from build123d import *

# Parameters (mm, degrees)
SKETCH_1_W      = 120
SKETCH_1_H      = 120
SKETCH_1_R      = 6.5
EXTRUDE_1_DEPTH = 10


with BuildPart() as part:
    # 草图1 → 凸台-拉伸1 (new body)
    with BuildSketch(Plane.XY):
        with Locations((60, 60)):
            Rectangle(SKETCH_1_W, SKETCH_1_H)
        with Locations((90, 35)):
            Circle(SKETCH_1_R, mode=Mode.SUBTRACT)
        with Locations((30, 85)):
            Circle(SKETCH_1_R, mode=Mode.SUBTRACT)
        with Locations((90, 85)):
            Circle(SKETCH_1_R, mode=Mode.SUBTRACT)
        with Locations((30, 35)):
            Circle(SKETCH_1_R, mode=Mode.SUBTRACT)
    extrude(amount=EXTRUDE_1_DEPTH)


solid = part.part
For this review, take the finished solid that the model builds, in its own axes (mm). Round coordinates to 2 decimals unless told otherwise and drop trailing zeros. Order: outer loops, then holes, each group sorted by start corner. A loop starts at its lowest first (then second) coordinate and runs counter-clockwise, first axis right, second up. Notation, with made-up numbers: (-27.75, 5.5) -> (7.25, 5.5) arc R27 cw to (7.25, 28.5) -> close; hole circle Ø5 at (43, -18). An arc over 180 degrees is marked (long way). Write item = value, one per line. Start each with the question number.
1) Take a section at C-C on z = 8. State the section outline as (x, y) points.
2) To check wall thickness, follow line 1 (Y direction, x = 30, z = 7.25); line 2 (Y direction, x = 84, z = 7); line 3 (X direction, y = 36.5, z = 8). State the ranges of each line that lie inside material, in increasing order. Write a range as from..to.
3) Take a section at A-A on x = 90. State the section outline as (y, z) points.
4) The part is to be moulded in two halves that separate along Y. For faces 1 (the face through (59, 0, 5)), 2 (the face through (28.591, 78.655, 4.93)), 3 (the face through (59, 120, 5)), say which applies: +Y half, -Y half, draft (parallel to the pull), parting line (faces both ways), or undercut.
5) Take a section at B-B on y = 85. State the section outline as (x, z) points, plus the area to 3 significant figures.
6) Insertion check: pin 1 (10.5 mm diameter, centred on x = 90, y = 85, fed in from -Z). The pin has a flat end and moves straight along its axis. Give the tip position at first contact, or say it passes through.
Verdict:
q1.outline = (0, 0) -> (120, 0) -> (120, 120) -> (0, 120) -> close; hole circle Ø13 at (30, 35); hole circle Ø13 at (30, 85); hole circle Ø13 at (90, 35); hole circle Ø13 at (90, 85)
q2.line_1 = 0..28.5, 41.5..78.5, 91.5..120
q2.line_2 = 0..32.5, 37.5..82.5, 87.5..120
q2.line_3 = 0..23.68, 36.32..83.68, 96.32..120
q3.outline = (0, 0) -> (28.5, 0) -> (28.5, 10) -> (0, 10) -> close; (41.5, 0) -> (78.5, 0) -> (78.5, 10) -> (41.5, 10) -> close; (91.5, 0) -> (120, 0) -> (120, 10) -> (91.5, 10) -> close
q4.face_1 = -Y half
q4.face_2 = undercut
q4.face_3 = +Y half
q5.outline = (0, 0) -> (23.5, 0) -> (23.5, 10) -> (0, 10) -> close; (36.5, 0) -> (83.5, 0) -> (83.5, 10) -> (36.5, 10) -> close; (96.5, 0) -> (120, 0) -> (120, 10) -> (96.5, 10) -> close
q5.area = 940 mm2
q6.pin_1 = through
